Input: part model. Units: mm. Frame: model coordinates. Give positions to 0.01 mm unless a question says otherwise; leave off trailing zeros. Loops run counter-clockwise (first coordinate to the right, second up) from the corner with the lowest first, then second, coordinate; pieces in that order, holes last. Notation, with made-up numbers: M -3,-3.5 L 37,-3.5 A19 cw 37,19.5 Z; hole C -18,1.25 d8. An arc over 180 degrees is marked long. One line per item, written item: value. Start each with the question number.
(1) Ray query, line 1 along X through (y, z) = (-50, 125.25); line 2 along X through (y, z) = (-46, 128.25); line 3 along Y through (x, z) = (-34, 129). Return the intervals inside material, ascending. Write a range as from..to.
(2) Section C-C on x = 17.5. Output: boundary loops of the cut face in (y, z) (3 decimals).
(3) Section A-A on y = -51. Output: boundary loops of the cut face in (x, z) (3 decimals), plus the area to 3 significant figures.
(4) Section B-B on z = 130.5. Output: boundary loops of the cut face in (x, y).
```python
from build123d import *

# Parameters (mm, degrees)
BOSS_EXTRUDE1_DEPTH = 9.525


with BuildPart() as part:
    # Sketch1 → Boss-Extrude1 (new body)
    with BuildSketch(Plane.XY.offset(133.35)):
        with BuildLine():
            Line((-76.2, -38.1), (-42.597094971, -38.1))
            ThreePointArc((-42.597094971, -38.1), (0, -57.15), (42.597094971, -38.1))
            Line((42.597094971, -38.1), (76.2, -38.1))
            Line((76.2, -38.1), (76.2, -114.3))
            Line((76.2, -114.3), (-76.2, -114.3))
            Line((-76.2, -114.3), (-76.2, -38.1))
        make_face()
    extrude(amount=-BOSS_EXTRUDE1_DEPTH)


solid = part.part
```
Output values:
1. line 1: x = -76.2..-27.68, 27.68..76.2
1. line 2: x = -76.2..-33.91, 33.91..76.2
1. line 3: y = -114.3..-45.94
2. outline: M -114.3,123.825 L -54.405,123.825 L -54.405,133.35 L -114.3,133.35 Z
3. outline: M -76.2,123.825 L -25.79,123.825 L -25.79,133.35 L -76.2,133.35 Z; M 25.79,123.825 L 76.2,123.825 L 76.2,133.35 L 25.79,133.35 Z
3. area: 960 mm²
4. outline: M -76.2,-114.3 L 76.2,-114.3 L 76.2,-38.1 L 42.6,-38.1 A57.15 cw -42.6,-38.1 L -76.2,-38.1 Z
